Can you work these out from the model? Positions are in its coordinate system, mm. A direction names the side the tool comes from. Round coordinates to 2 decimals unless told otherwise and drop trailing zeros. Loops run counter-clockwise (first coordinate to the right, second up) from the corner with the lowest first, then second, coordinate; pieces in that order, holes last. Notation, with made-up numbers: M 76,36.5 L 123,36.5 A21 cw 123,68.5 Z; hole C 14.25,-39.75 d7. An arc over 180 degrees is marked long. Return JSON: item names as keys, results as strings.
```python
from build123d import *

# Parameters (mm, degrees)
SKETCH1_W           = 112
SKETCH1_H           = 27
BOSS_EXTRUDE1_DEPTH = 2
SKETCH2_R           = 1.6
CUT_EXTRUDE1_DEPTH  = 58.638962517
FILLET1_R           = 2
SKETCH3_R           = 1.6
CUT_EXTRUDE2_DEPTH  = 2


with BuildPart() as part:
    # Sketch1 → Boss-Extrude1 (new body)
    with BuildSketch(Plane(origin=(0, 0, 0), x_dir=(1, 0, 0), z_dir=(0, 1, 0))):
        Rectangle(SKETCH1_W, SKETCH1_H)
    extrude(amount=BOSS_EXTRUDE1_DEPTH)

    # Sketch2 → Cut-Extrude1 (cut, through all)
    with BuildSketch(Plane(origin=(0, 2, 0), x_dir=(1, 0, 0), z_dir=(0, 1, 0))):
        with Locations(Location((-52, 10, 0), (0, 0, 270))):
            Circle(SKETCH2_R)
        with Locations(Location((52, 10, 0), (0, 0, 270))):
            Circle(SKETCH2_R)
        with Locations(Location((52, -10, 0), (0, 0, 270))):
            Circle(SKETCH2_R)
        with Locations(Location((-52, -10, 0), (0, 0, 270))):
            Circle(SKETCH2_R)
    extrude(amount=-CUT_EXTRUDE1_DEPTH, mode=Mode.SUBTRACT)

    # Fillet1
    fillet1_edges = [part.edges().sort_by_distance(p)[0] for p in [
        (56, 1, 13.5),
        (-56, 1, 13.5),
        (-56, 1, -13.5),
        (56, 1, -13.5),
    ]]
    fillet(fillet1_edges, radius=FILLET1_R)

    # Sketch3 → Cut-Extrude2 (cut)
    with BuildSketch(Plane(origin=(0, 2, 0), x_dir=(1, 0, 0), z_dir=(0, 1, 0))):
        with BuildLine():
            Line((1.637186959, -6.05), (37.362813041, -6.05))
            ThreePointArc((37.362813041, -6.05), (38.905503304, -5.488506663), (39.726351648, -4.066755626))
            Line((39.726351648, -4.066755626), (41.013538607, 3.233244374))
            ThreePointArc((41.013538607, 3.233244374), (40.488506663, 5.192690263), (38.65, 6.05))
            Line((38.65, 6.05), (0.35, 6.05))
            ThreePointArc((0.35, 6.05), (-1.488506663, 5.192690263), (-2.013538607, 3.233244374))
            Line((-2.013538607, 3.233244374), (-0.726351648, -4.066755626))
            ThreePointArc((-0.726351648, -4.066755626), (0.094496696, -5.488506663), (1.637186959, -6.05))
        make_face()
        with BuildLine():
            Line((-23.5, 6.05), (-39.5, 6.05))
            ThreePointArc((-39.5, 6.05), (-41.338506663, 5.192690263), (-41.863538607, 3.233244374))
            Line((-41.863538607, 3.233244374), (-40.576351648, -4.066755626))
            ThreePointArc((-40.576351648, -4.066755626), (-39.755503304, -5.488506663), (-38.212813041, -6.05))
            Line((-38.212813041, -6.05), (-24.787186959, -6.05))
            ThreePointArc((-24.787186959, -6.05), (-23.244496696, -5.488506663), (-22.423648352, -4.066755626))
            Line((-22.423648352, -4.066755626), (-21.136461393, 3.233244374))
            ThreePointArc((-21.136461393, 3.233244374), (-21.661493337, 5.192690263), (-23.5, 6.05))
        make_face()
        with Locations(Location((-43.995, 0, 0), (0, 0, 270))):
            Circle(SKETCH3_R)
        with Locations(Location((-19.005, 0, 0), (0, 0, 270))):
            Circle(SKETCH3_R)
        with Locations(Location((-4.02, 0, 0), (0, 0, 270))):
            Circle(SKETCH3_R)
        with Locations(Location((43.02, 0, 0), (0, 0, 270))):
            Circle(SKETCH3_R)
    extrude(amount=-CUT_EXTRUDE2_DEPTH, mode=Mode.SUBTRACT)


solid = part.part
```
Q1. Suppose I cut it at D-D, the plane z = 0. Please give me the cut outline in (x, y) (3 decimals).
Results:
{"outline": "M -56,0 L -45.595,0 L -45.595,2 L -56,2 Z; M -42.395,0 L -41.293,0 L -41.293,2 L -42.395,2 Z; M -21.707,0 L -20.605,0 L -20.605,2 L -21.707,2 Z; M -17.405,0 L -5.62,0 L -5.62,2 L -17.405,2 Z; M -2.42,0 L -1.443,0 L -1.443,2 L -2.42,2 Z; M 40.443,0 L 41.42,0 L 41.42,2 L 40.443,2 Z; M 44.62,0 L 56,0 L 56,2 L 44.62,2 Z"}
Q2. Suppose I cut it at C-C, the plane y = 0.4. State how many separate pieces and enclosed holes the cut face has, plus the area to 3 significant figures.
Results:
{"separate pieces": "1", "enclosed holes": "10", "area": "2,220 mm2"}
Q3. Thinking about a two-plate mould opening in Z: for faces 3 (the flat face through (-1, 1, 13.5)), 4 (the cylindrical face through (-21.643, 1.014, -5.17)), 5 (the cylindrical face through (55.4, 1.01, -12.93)), 6 (the flat face through (-1, 2, -6)), which applies, pulls with the +Z half, pulls with the -Z half, needs draft (parallel to the pull), parting line crosses it, or undercut?
Results:
{"face 3": "pulls with the +Z half", "face 4": "undercut", "face 5": "pulls with the -Z half", "face 6": "needs draft"}
Q4. If I drill on line 1 along X through (y, z) = (1.3, -10.25); line 2 along X through (y, z) = (1.15, -3.5); line 3 along Z through (x, y) = (5, 0.25), over which ranges is the centre line in solid material (lowest first)?
Results:
{"line 1": "x = -56 to -53.58, -50.42 to 50.42, 53.58 to 56", "line 2": "x = -56 to -41.9, -21.1 to -2.05, 41.05 to 56", "line 3": "z = -13.5 to -6.05, 6.05 to 13.5"}
Q5. Suppose I cut it at B-B, the plane x = 35. Please give me the cut outline in (y, z).
Results:
{"outline": "M 0,-13.5 L 2,-13.5 L 2,-6.05 L 0,-6.05 Z; M 0,6.05 L 2,6.05 L 2,13.5 L 0,13.5 Z"}
Q6. On a 3-axis mill with a long thin cutter (end or side, diameter ignored), from which of +Z, -Z, +X, -X, +Y, -Y can I reach the whole of each face in a straight line? I mean faces 1 (the cylindrical face through (55.4, 1.01, 12.93)), 2 (the cylindrical face through (-23.26, 1.01, 5.5)). Say none if no direction works.
Results:
{"face 1": "+Z, +X, +Y, -Y", "face 2": "+Y, -Y"}
Q7. Suppose I cut it at A-A, the plane z = 10. Please give me the cut outline in (x, y).
Results:
{"outline": "M -56,0 L -53.6,0 L -53.6,2 L -56,2 Z; M -50.4,0 L 50.4,0 L 50.4,2 L -50.4,2 Z; M 53.6,0 L 56,0 L 56,2 L 53.6,2 Z"}
